Work out the finished part from the listing and answer in its coordinate system (mm). Round coordinates to 2 decimals unless told otherwise and drop trailing zeros. Order: outer loops, then holes, each group sorted by start corner. A loop starts at its lowest first (then second) coordinate and runs counter-clockwise, first axis right, second up. Notation, with made-up numbers: (74, 89.25) -> (125, 89.25) arc R27 ccw to (125, 116.25) -> close; hole circle Ø1 at (42.25, -26). An arc over 180 degrees is marked (long way). Use one line per item in the form item = value.
```python
from build123d import *

# Parameters (mm, degrees)
SKETCH2_R = 3.25


with BuildPart() as part:
    # Sweep1: sweep along a path in Sketch1
    with BuildLine(Plane.XY) as sweep1_path:
        Line((0, 0), (0, 1193))
        ThreePointArc((0, 1193), (12.30151519, 1222.69848481), (42, 1235))
        Line((42, 1235), (2100, 1235))
        ThreePointArc((2100, 1235), (2129.69848481, 1222.69848481), (2142, 1193))
        Line((2142, 1193), (2142, 985))
    # Sketch2 → Sweep1 (sweep)
    with BuildSketch(Plane(origin=(0, 0, 0), x_dir=(1, 0, 0), z_dir=(0, 1, 0))):
        Circle(SKETCH2_R)
    sweep(path=sweep1_path.line)


solid = part.part
```
Item 1: Flat-ended cylindrical pins translate along their axes: P1, Ø1, axis at y = 857.5, z = 0.5, coming from the +X side; P2, Ø2, axis at x = 2142.5, z = -0.5, coming from the -Y side; P3, Ø1, axis at y = 365, z = 2, coming from the -X side. Find the tip coordinate at first contact, or state that the pin passes through.
Findings:
P1 = 3.25
P2 = 985
P3 = -2.88
Item 2: The part is cut by section B-B, the plane y = 1132.5. Give the vertices of the cut face in (x, z), and give its area (3 significant figures).
Findings:
outline = circle Ø6.5 at (0, 0); circle Ø6.5 at (2142, 0)
area = 66.4 mm^2
Item 3: The part is cut by section C-C, the plane x = 215.5. Give the vertices of the cut face in (y, z), and give its area (3 significant figures).
Findings:
outline = circle Ø6.5 at (1235, 0)
area = 33.2 mm^2
Item 4: The part is cut by section D-D, the plane y = 634.5. Give the vertices of the cut face in (x, z).
Findings:
outline = circle Ø6.5 at (0, 0)
Item 5: The part is cut by section A-A, the plane z = 0. Give the vertices of the cut face in (x, y), and give its area (3 significant figures).
Findings:
outline = (-3.25, 0) -> (3.25, 0) -> (3.25, 1193) arc R38.75 cw to (42, 1231.75) -> (2100, 1231.75) arc R38.75 cw to (2138.75, 1193) -> (2138.75, 985) -> (2145.25, 985) -> (2145.25, 1193) arc R45.25 ccw to (2100, 1238.25) -> (42, 1238.25) arc R45.25 ccw to (-3.25, 1193) -> close
area = 23,300 mm^2
Item 6: Consider line 1 along X through (y, z) = (1062.5, 1); line 2 along X through (y, z) = (80, 0.25); line 3 along Y through (x, z) = (1694.5, -0.75). Determine where each line is inside the solid, lowest interval first.
Findings:
line_1 = -3.09 to 3.09, 2138.91 to 2145.09
line_2 = -3.24 to 3.24
line_3 = 1231.84 to 1238.16
